Check sheet for the drawn part. Datum: minimum x, y, z corner. Units: mm. A direction names the side the tool comes from. Give positions to 0.01 mm unless a question says otherwise; leave off trailing zeros. Write each loop counter-clockwise with the first axis right and the second up, starting at its lowest first coordinate (ties: lowest second). Pieces come first, ordered by that corner, then holes. Notation, with made-up numbers: M 32.5,-9.5 L 39.5,-9.5 A30 ccw 39.5,18.5 Z; hole C 14,-13.5 d3. An arc over 180 degrees is marked long. Use CSV: the item, a comma, the result in double quotes. Start each with the question number.
1. Cross-section at C-C, the plane z = 23.5. Enter the section's corners in (x, y).
2. Cross-section at B-B, the plane x = 13.5. Enter the section's corners in (y, z) (1 decimal).
3. Depth check by flat-ended pin: P1, Ø5, axis at y = 11, z = 31, coming from the -X side; P2, Ø1.5, axis at y = 3, z = 22, coming from the -X side; P3, Ø5, axis at x = 12.5, z = 10, coming from the +Y side; P4, Ø1.5, axis at y = 4.5, z = 21, coming from the +X side (1 decimal). Enter the tip coordinate at first touch or a pass-through.
4. Access from +Z, -Z, +X, -X, +Y, -Y to the whole of each face (thin tool, end or side, straight path). Record for the marked faces 1 and 2.
5. Scan lines: line 1 (Z direction, x = 15.25, y = 11.5); line 2 (Y direction, x = 5, z = 17); line 3 (X direction, y = 12.75, z = 27). Record each from-to range of solid material in increasing order.
6. Cross-section at A-A, the plane z = 3. Enter the section's corners in (x, y) (1 decimal), and give its area (3 significant figures).
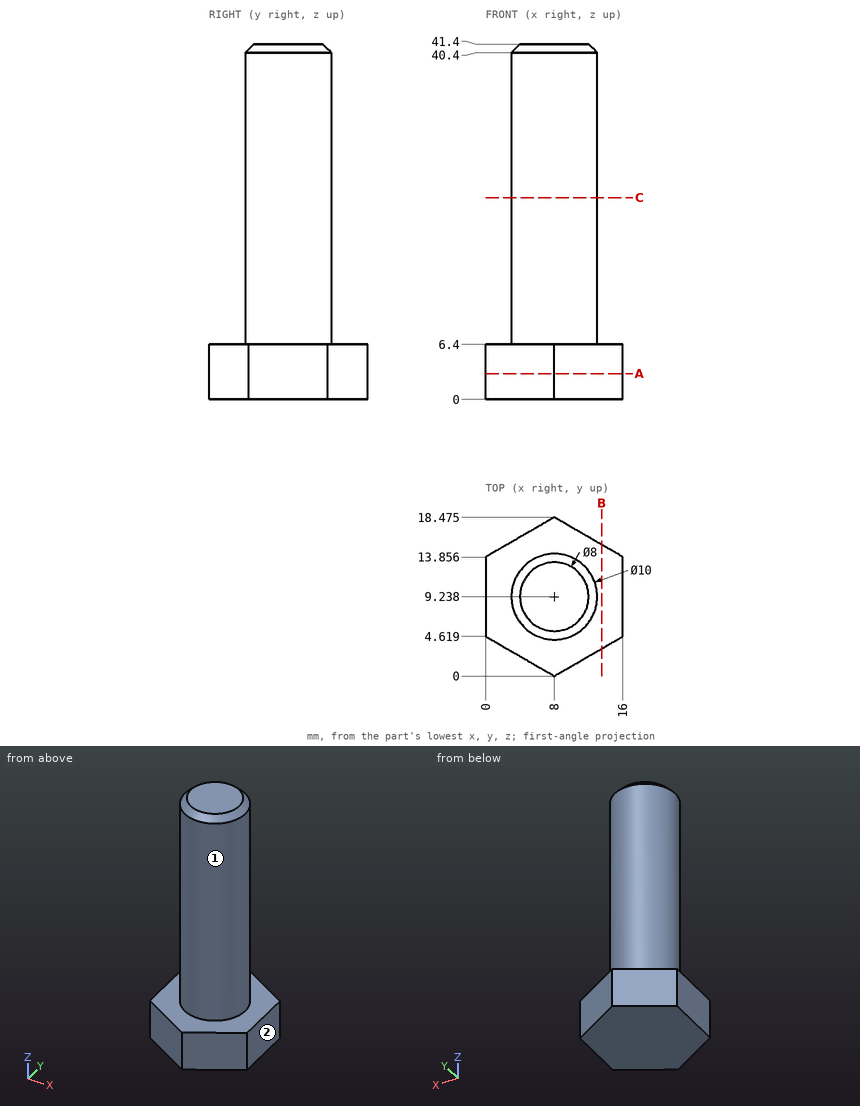
Worked answers:
1,outline,"C 8,9.24 d10"
2,outline,"M 3.2,0 L 15.3,0 L 15.3,6.4 L 3.2,6.4 Z"
3,P1,"stops at x = 3"
3,P2,"passes through"
3,P3,"stops at y = 13.82"
3,P4,"stops at x = 11"
4,face 1,"+Z"
4,face 2,"+Z, -Z, +X, +Y, -Y"
5,line 1,"z = 0 to 6.4"
5,line 2,"y = 5.24 to 13.24"
5,line 3,"x = 4.44 to 11.56"
6,outline,"M 0,4.6 L 8,0 L 16,4.6 L 16,13.9 L 8,18.5 L 0,13.9 Z"
6,area,"222 mm^2"
